Job drawing, mm, ordinate dimensions from the low corner. One solid piece. Round coordinates to 2 decimals unless told otherwise and drop trailing zeros. Loops run counter-clockwise (first coordinate to the right, second up) from the corner with the lowest first, then second, coordinate; pieces in that order, holes last. Notation, with made-up numbers: M 19,-21 L 52,-21 A18 cw 52,-15 Z; hole C -16.75,-14.5 d5. An arc over 180 degrees is marked long. Use a Markdown table: item, result. Add a question column.
(1) Wall check: L1, parallel to Z at x = 18.5, y = 25; L2, parallel to X at y = 44, z = 37. Give the ranges that are in metal, low to high.
(2) Band-saw the part on A-A, the plane y = 25. Write the cut outline in (x, z), and give its area (3 significant figures).
(3) Flat gauge pins, fed straight in: P1, Ø10, axis at y = 20.5, z = 23.5, coming from the +X side; P2, Ø2, axis at x = 20.5, z = 12.5, coming from the -Y side; P3, Ø1, axis at x = 7.5, y = 20, coming from the +Z side; P4, Ø1, axis at y = 25, z = 44.5, coming from the -X side. Where does each tip first touch, or does it go through?
(4) Two-plate mould, pull along Z, no slides. Class the marked faces 1, 2 and 3: released by +Z, released by -Z, zero draft, split by the parting line, or undercut.
(5) Band-saw the part on C-C, the plane x = 5. Write the cut outline in (y, z), and give its area (3 significant figures).
(6) Band-saw the part on D-D, the plane y = 12. Write the cut outline in (x, z), and give its area (3 significant figures).
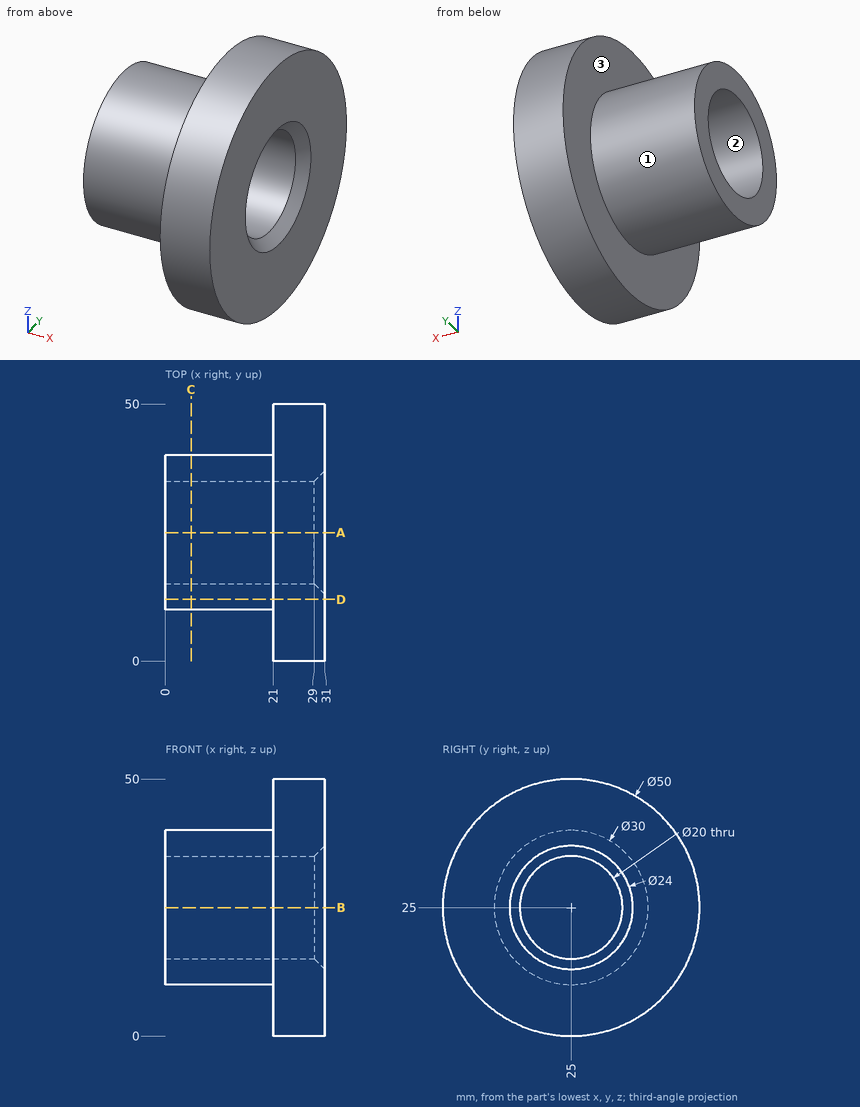
Return value:
| question | item | result |
|---|---|---|
| 1 | L1 | 10 to 15, 35 to 40 |
| 1 | L2 | 21 to 31 |
| 2 | outline | M 0,10 L 21,10 L 21,0 L 31,0 L 31,13 L 29,15 L 0,15 Z; M 0,35 L 29,35 L 31,37 L 31,50 L 21,50 L 21,40 L 0,40 Z |
| 2 | area | 506 mm^2 |
| 3 | P1 | through |
| 3 | P2 | y = 2.87 |
| 3 | P3 | z = 39.31 |
| 3 | P4 | x = 21 |
| 4 | face 1 | split by the parting line |
| 4 | face 2 | undercut |
| 4 | face 3 | zero draft |
| 5 | outline | C 25,25 d30; hole C 25,25 d20 |
| 5 | area | 393 mm^2 |
| 6 | outline | M 0,17.52 L 21,17.52 L 21,3.65 L 31,3.65 L 31,46.35 L 21,46.35 L 21,32.48 L 0,32.48 Z |
| 6 | area | 741 mm^2 |
